```python
from build123d import *

# Parameters (mm, degrees)
SKETCH2_W           = 80
SKETCH2_H           = 126
SKETCH2_R           = 19
BOSS_EXTRUDE1_DEPTH = 68.5


with BuildPart() as part:
    # Sketch2 → Boss-Extrude1 (new, symmetric)
    with BuildSketch(Plane(origin=(0, 0, 0), x_dir=(1, 0, 0), z_dir=(0, 1, 0))):
        Rectangle(SKETCH2_W, SKETCH2_H)
        with Locations(Location((0, 34, 0), (0, 0, 270))):
            Circle(SKETCH2_R, mode=Mode.SUBTRACT)
        with Locations(Location((0, -34, 0), (0, 0, 270))):
            Circle(SKETCH2_R, mode=Mode.SUBTRACT)
    extrude(amount=BOSS_EXTRUDE1_DEPTH, both=True)


solid = part.part
```
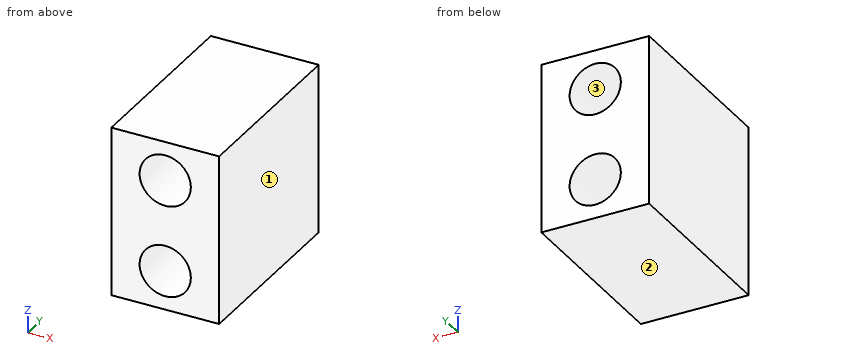
Input: part model. Units: mm. Frame: model coordinates. Face numbers are marked on the shaded views. Coordinates: 2 decimals unless noted, no trailing zeros. Write each loop counter-clockwise with the first axis right and the second up, starting at its lowest first coordinate (ties: lowest second). Pieces come first, ordered by that corner, then holes. Notation, with made-up numbers: M 70.25,41 L 113.25,41 A10 cw 113.25,58 Z; hole C 44.5,3 d7. An arc over 180 degrees is marked long. Use one line per item in the form item = value.
Q1. Draft query along X for the marked faces 1, 2 and 3. Return one class per face: released by +X, released by -X, zero draft, split by the parting line, or undercut.
Answer below:
face_1 = released by +X
face_2 = zero draft
face_3 = undercut
Q2. Material intervals for probe 1 along X at (y, z) = (15, 34); probe 2 along Z at (x, y) = (2, 52); probe 3 along Z at (x, y) = (11, -47), sorted ascending. Write a range as from..to.
Answer below:
probe_1 = -40..-19, 19..40
probe_2 = -63..-52.89, -15.11..15.11, 52.89..63
probe_3 = -63..-49.49, -18.51..18.51, 49.49..63
Q3. Section B-B (z = 44.5). Return loops of the section in (x, y).
Answer below:
outline = M -40,-68.5 L -15.84,-68.5 L -15.84,68.5 L -40,68.5 Z; M 15.84,-68.5 L 40,-68.5 L 40,68.5 L 15.84,68.5 Z
Q4. Section A-A (x = 0). Return loops of the section in (y, z).
Answer below:
outline = M -68.5,-63 L 68.5,-63 L 68.5,-53 L -68.5,-53 Z; M -68.5,-15 L 68.5,-15 L 68.5,15 L -68.5,15 Z; M -68.5,53 L 68.5,53 L 68.5,63 L -68.5,63 Z
Q5. Section C-C (y = -18). Return loops of the section in (x, z).
Answer below:
outline = M -40,-63 L 40,-63 L 40,63 L -40,63 Z; hole C 0,-34 d38; hole C 0,34 d38
Q6. Section D-D (z = -34). Return loops of the section in (x, y), plus the area to 3 significant figures.
Answer below:
outline = M -40,-68.5 L -19,-68.5 L -19,68.5 L -40,68.5 Z; M 19,-68.5 L 40,-68.5 L 40,68.5 L 19,68.5 Z
area = 5,750 mm²
